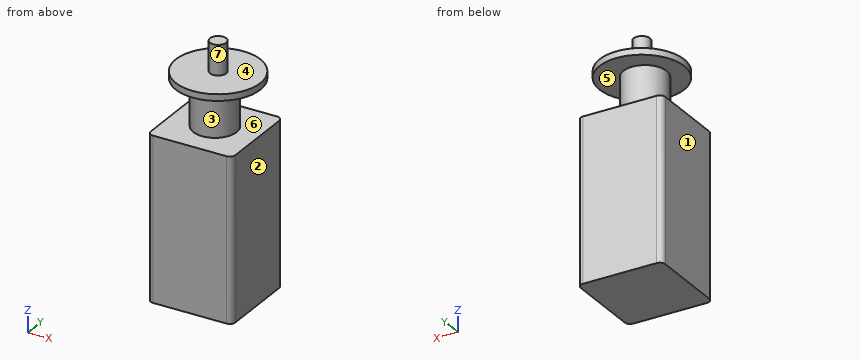
```python
from build123d import *

# Parameters (mm, degrees)
SKETCH1_W           = 156
SKETCH1_H           = 156
BOSS_EXTRUDE1_DEPTH = 300
SKETCH2_R           = 40
BOSS_EXTRUDE2_DEPTH = 88
SKETCH3_R           = 78
BOSS_EXTRUDE3_DEPTH = 12
FILLET1_R           = 10
SKETCH4_R           = 15
BOSS_EXTRUDE4_DEPTH = 55


with BuildPart() as part:
    # Sketch1 → Boss-Extrude1 (new body)
    with BuildSketch(Plane.XY):
        with Locations((78, 78)):
            Rectangle(SKETCH1_W, SKETCH1_H)
    extrude(amount=BOSS_EXTRUDE1_DEPTH)

    # Sketch2 → Boss-Extrude2 (add)
    with BuildSketch(Plane.XY.offset(300)):
        with Locations(Location((78, 78, 0), (0, 0, 180))):
            Circle(SKETCH2_R)
    extrude(amount=BOSS_EXTRUDE2_DEPTH)

    # Sketch3 → Boss-Extrude3 (add)
    with BuildSketch(Plane.XY.offset(388)):
        with Locations((83.788071994, 78)):
            Circle(SKETCH3_R)
    extrude(amount=BOSS_EXTRUDE3_DEPTH)

    # Fillet1
    fillet1_edges = [part.edges().sort_by_distance(p)[0] for p in [
        (0, 156, 150),
        (156, 156, 150),
        (156, 0, 150),
        (0, 0, 150),
    ]]
    fillet(fillet1_edges, radius=FILLET1_R)

    # Sketch4 → Boss-Extrude4 (add)
    with BuildSketch(Plane.XY.offset(400)):
        with Locations((83.788071994, 78)):
            Circle(SKETCH4_R)
    extrude(amount=BOSS_EXTRUDE4_DEPTH)


solid = part.part
```
Source: CAD feature listing. Evaluate the final solid. Frame: model axes, mm. Face numbers are marked on the shaded views. A direction names the side the tool comes from. Coordinates: 2 decimals unless noted, no trailing zeros. Write each loop counter-clockwise with the first axis right and the second up, starting at its lowest first coordinate (ties: lowest second). Pieces come first, ordered by that corner, then holes. Notation, with made-up numbers: M -19,85 L -1,85 A8 cw -1,94 Z; hole C -17,-34 d3. An arc over 180 degrees is marked long. Answer as a JSON object with one key per item and string values.
1. Draft query along Z for the marked faces 4, 5, 6 and 7. Return one class per face: released by +Z, released by -Z, zero draft, split by the parting line, or undercut.
Evaluation:
{"face 4": "released by +Z", "face 5": "undercut", "face 6": "undercut", "face 7": "zero draft"}
2. Cut plane A-A on x = 137. Output: boundary loops of the cut face in (y, z).
Evaluation:
{"outline": "M 0,0 L 156,0 L 156,300 L 0,300 Z; M 20.97,388 L 135.03,388 L 135.03,400 L 20.97,400 Z"}
3. Cut plane B-B on y = 78. Output: boundary loops of the cut face in (x, z), plus the area to 3 significant figures.
Evaluation:
{"outline": "M 0,0 L 156,0 L 156,300 L 118,300 L 118,388 L 161.79,388 L 161.79,400 L 98.79,400 L 98.79,455 L 68.79,455 L 68.79,400 L 5.79,400 L 5.79,388 L 38,388 L 38,300 L 0,300 Z", "area": "57,400 mm^2"}
4. Access query for the marked faces 1, 2 and 3. Directions: +Z, -Z, +X, -X, +Y, -Y. A direction counts if a zero-diameter tool reaches every point of the face in a straight line with its end or side. Return the directions, or none.
Evaluation:
{"face 1": "+Z, -Z, -X, +Y, -Y", "face 2": "-Z, +X, +Y, -Y", "face 3": "none"}
5. Contact query for flat-ended pins moving along their axis: P1, Ø10, axis at x = 42, z = 313.5, coming from the +Y side; P2, Ø5, axis at x = 99, y = 94, coming from the +Z side; P3, Ø8, axis at x = 124.5, z = 353, coming from the +Y side; P4, Ø3, axis at y = 109, z = 64, coming from the +X side. Output: stop coordinate, or through.
Evaluation:
{"P1": "y = 103.28", "P2": "z = 400", "P3": "through", "P4": "x = 156"}
6. Cut plane C-C on z = 253. Output: boundary loops of the cut face in (x, y).
Evaluation:
{"outline": "M 0,10 A10 ccw 10,0 L 146,0 A10 ccw 156,10 L 156,146 A10 ccw 146,156 L 10,156 A10 ccw 0,146 Z"}
7. Ray query, L1, parallel to Z at x = 58.5, y = 139.5; L2, parallel to X at y = 128, z = 33.5; L3, parallel to Z at x = 89, y = 95. Return the intervals inside material, ascending.
Evaluation:
{"L1": "0 to 300, 388 to 400", "L2": "0 to 156", "L3": "0 to 400"}
8. Cut plane D-D on y = 130. Output: boundary loops of the cut face in (x, z), plus the area to 3 significant figures.
Evaluation:
{"outline": "M 0,0 L 156,0 L 156,300 L 0,300 Z; M 25.65,388 L 141.93,388 L 141.93,400 L 25.65,400 Z", "area": "48,200 mm^2"}
